```python
from build123d import *

# Parameters (mm, degrees)
SKETCH_1_R          = 4.1077368
SKETCH_1_W          = 5
SKETCH_1_H          = 5
EXTRUDE_1_DEPTH     = 2720
SKETCH_2_W          = 4
SKETCH_2_H          = 5
CUT_EXTRUDE_1_DEPTH = 2721.827080136
SKETCH_3_W          = 4
SKETCH_3_H          = 11
CUT_EXTRUDE_2_DEPTH = 2721.827080136


with BuildPart() as part:
    # 草图1 → 拉伸1 (new body)
    with BuildSketch(Plane.XY):
        with BuildLine():
            Line((12.5, 0), (12.5, -2))
            Line((12.5, -2), (9.5, -2))
            Line((9.5, -2), (9.5, -7))
            ThreePointArc((9.5, -7), (15, -8.308258509), (20.5, -7))
            Line((20.5, -7), (20.5, -2))
            Line((20.5, -2), (17.5, -2))
            Line((17.5, -2), (17.5, 0))
            Line((17.5, 0), (42.5, 0))
            Line((42.5, 0), (42.5, -2))
            Line((42.5, -2), (39.5, -2))
            Line((39.5, -2), (39.5, -7))
            ThreePointArc((39.5, -7), (45, -8.308258509), (50.5, -7))
            Line((50.5, -7), (50.5, -2))
            Line((50.5, -2), (47.5, -2))
            Line((47.5, -2), (47.5, 0))
            Line((47.5, 0), (60, 0))
            Line((60, 0), (60, -12.5))
            Line((60, -12.5), (58, -12.5))
            Line((58, -12.5), (58, -9.5))
            Line((58, -9.5), (53, -9.5))
            ThreePointArc((53, -9.5), (51.691741491, -15), (53, -20.5))
            Line((53, -20.5), (58, -20.5))
            Line((58, -20.5), (58, -17.5))
            Line((58, -17.5), (60, -17.5))
            Line((60, -17.5), (60, -30))
            Line((60, -30), (47.5, -30))
            Line((47.5, -30), (47.5, -28))
            Line((47.5, -28), (50.5, -28))
            Line((50.5, -28), (50.5, -23))
            ThreePointArc((50.5, -23), (45, -21.691741491), (39.5, -23))
            Line((39.5, -23), (39.5, -28))
            Line((39.5, -28), (42.5, -28))
            Line((42.5, -28), (42.5, -30))
            Line((42.5, -30), (17.5, -30))
            Line((17.5, -30), (17.5, -28))
            Line((17.5, -28), (20.5, -28))
            Line((20.5, -28), (20.5, -23))
            ThreePointArc((20.5, -23), (15, -21.691741491), (9.5, -23))
            Line((9.5, -23), (9.5, -28))
            Line((9.5, -28), (12.5, -28))
            Line((12.5, -28), (12.5, -30))
            Line((12.5, -30), (0, -30))
            Line((0, -30), (0, -17.5))
            Line((0, -17.5), (2, -17.5))
            Line((2, -17.5), (2, -20.5))
            Line((2, -20.5), (7, -20.5))
            ThreePointArc((7, -20.5), (8.308258509, -15), (7, -9.5))
            Line((7, -9.5), (2, -9.5))
            Line((2, -9.5), (2, -12.5))
            Line((2, -12.5), (0, -12.5))
            Line((0, -12.5), (0, 0))
            Line((0, 0), (12.5, 0))
        make_face()
        with Locations((15, -15)):
            Circle(SKETCH_1_R, mode=Mode.SUBTRACT)
        with Locations(Location((45, -15, 0), (0, 0, 180))):
            Circle(SKETCH_1_R, mode=Mode.SUBTRACT)
        with BuildLine():
            Line((32, -12.5), (28, -12.5))
            Line((28, -12.5), (28, -9.5))
            Line((28, -9.5), (23, -9.5))
            ThreePointArc((23, -9.5), (21.691741491, -15), (23, -20.5))
            Line((23, -20.5), (28, -20.5))
            Line((28, -20.5), (28, -17.5))
            Line((28, -17.5), (32, -17.5))
            Line((32, -17.5), (32, -20.5))
            Line((32, -20.5), (37, -20.5))
            ThreePointArc((37, -20.5), (38.308258509, -15), (37, -9.5))
            Line((37, -9.5), (32, -9.5))
            Line((32, -9.5), (32, -12.5))
        make_face(mode=Mode.SUBTRACT)
        with Locations((55.5, -4.5)):
            Rectangle(SKETCH_1_W, SKETCH_1_H, mode=Mode.SUBTRACT)
        with Locations((25.5, -25.5)):
            Rectangle(SKETCH_1_W, SKETCH_1_H, mode=Mode.SUBTRACT)
        with Locations((25.5, -4.5)):
            Rectangle(SKETCH_1_W, SKETCH_1_H, mode=Mode.SUBTRACT)
        with Locations((4.5, -25.5)):
            Rectangle(SKETCH_1_W, SKETCH_1_H, mode=Mode.SUBTRACT)
        with Locations((4.5, -4.5)):
            Rectangle(SKETCH_1_W, SKETCH_1_H, mode=Mode.SUBTRACT)
        with Locations((55.5, -25.5)):
            Rectangle(SKETCH_1_W, SKETCH_1_H, mode=Mode.SUBTRACT)
        with Locations((34.5, -25.5)):
            Rectangle(SKETCH_1_W, SKETCH_1_H, mode=Mode.SUBTRACT)
        with Locations((34.5, -4.5)):
            Rectangle(SKETCH_1_W, SKETCH_1_H, mode=Mode.SUBTRACT)
    extrude(amount=EXTRUDE_1_DEPTH)

    # 草图2 → 切除-拉伸1 (cut, through all)
    with BuildSketch(Plane.XY.offset(2720)):
        with Locations((30, -4.5)):
            Rectangle(SKETCH_2_W, SKETCH_2_H)
        with Locations((30, -25.5)):
            Rectangle(SKETCH_2_W, SKETCH_2_H)
    extrude(amount=-CUT_EXTRUDE_1_DEPTH, mode=Mode.SUBTRACT)

    # 草图3 → 切除-拉伸2 (cut, through all)
    with BuildSketch(Plane.XY.offset(2720)):
        with Locations((30, -15)):
            Rectangle(SKETCH_3_W, SKETCH_3_H)
    extrude(amount=-CUT_EXTRUDE_2_DEPTH, mode=Mode.SUBTRACT)


solid = part.part
```
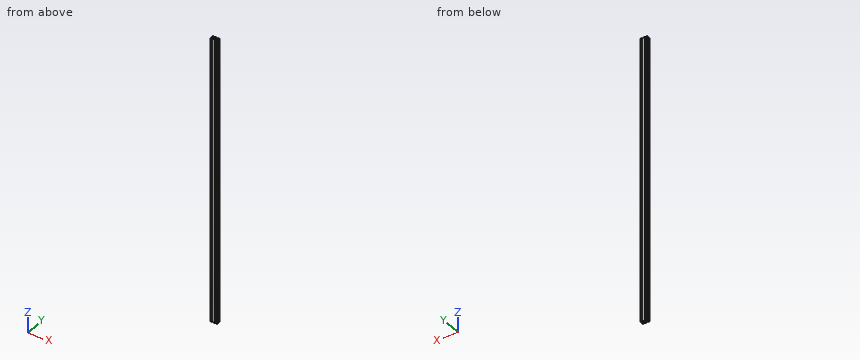
Verification items for the finished model (mm, model axes). Coordinates: 2 decimals unless noted, no trailing zeros. Put each result on its own line as item: value. Start each with the question number.
1) Material ranges on L1, parallel to Y at x = 34, z = 273; L2, parallel to Y at x = 10.5, z = 1789; L3, parallel to X at y = -25.5, z = 2254, recorded low to high.
2) Cross-section at A-A (z = 266). State how many separate pieces and enclosed holes the cut face has, plus the area to 3 significant figures.
3) Go/stop test with flat-tipped pins: pin 1 (5 mm diameter, centred on y = -11.5, z = 1611.5, fed in from -X); pin 2 (2 mm diameter, centred on x = 33.5, y = -26, fed in from +Z). Record where each tip stops, or that it passes through.
Geometry check:
1. L1: y = -30 to -28, -23 to -20.5, -9.5 to -7, -2 to 0
1. L2: y = -30 to -28, -22.55 to -7.45, -2 to 0
1. L3: x = 0 to 2, 7 to 9.5, 20.5 to 23, 37 to 39.5, 50.5 to 53, 58 to 60
2. separate pieces: 1
2. enclosed holes: 9
2. area: 832 mm^2
3. pin 1: stops at x = 0
3. pin 2: passes through
